Geometry: final body of the model. Coordinates: model frame, mm. Face numbers are marked on the shaded views. Round coordinates to 2 decimals unless told otherwise and drop trailing zeros. Write each loop counter-clockwise with the first axis right and the second up, starting at its lowest first coordinate (ties: lowest second). Pieces come first, ordered by that corner, then holes. Notation, with made-up numbers: (-33.5, 8.5) - (-9.5, 8.5) arc R17 cw to (-9.5, 28.5) - close; hole circle Ø9 at (15, -35.5). An arc over 180 degrees is marked (long way). Write each question's results on one line, items separated by ' | '.
from build123d import *

# Parameters (mm, degrees)
SKETCH_1_W          = 268
SKETCH_1_H          = 150
EXTRUDE_1_DEPTH     = 12
SKETCH_2_W          = 258
SKETCH_2_H          = 150
CUT_EXTRUDE_1_DEPTH = 2
CUT_EXTRUDE_2_DEPTH = 154.886321679
HOLE_WIZARD_M6_1_D  = 5
CHAMFER_1_SIZE      = 3


with BuildPart() as part:
    # 草图1 → 凸台-拉伸1 (new body)
    with BuildSketch(Plane.XY):
        Rectangle(SKETCH_1_W, SKETCH_1_H)
    extrude(amount=EXTRUDE_1_DEPTH)

    # 草图2 → 切除-拉伸1 (cut)
    with BuildSketch(Plane.XY.offset(12)):
        Rectangle(SKETCH_2_W, SKETCH_2_H)
    extrude(amount=-CUT_EXTRUDE_1_DEPTH, mode=Mode.SUBTRACT)

    # 草图3 → 切除-拉伸2 (cut, through all)
    with BuildSketch(Plane.XY.offset(10)):
        with BuildLine():
            Line((-80, 53.3), (-50, 53.3))
            ThreePointArc((-50, 53.3), (-46.7, 50), (-50, 46.7))
            Line((-50, 46.7), (-80, 46.7))
            ThreePointArc((-80, 46.7), (-83.3, 50), (-80, 53.3))
        make_face()
        with BuildLine():
            Line((50, 53.3), (80, 53.3))
            ThreePointArc((80, 53.3), (83.3, 50), (80, 46.7))
            Line((80, 46.7), (50, 46.7))
            ThreePointArc((50, 46.7), (46.7, 50), (50, 53.3))
        make_face()
        with BuildLine():
            Line((-80, -46.7), (-50, -46.7))
            ThreePointArc((-50, -46.7), (-46.7, -50), (-50, -53.3))
            Line((-50, -53.3), (-80, -53.3))
            ThreePointArc((-80, -53.3), (-83.3, -50), (-80, -46.7))
        make_face()
        with BuildLine():
            Line((50, -46.7), (80, -46.7))
            ThreePointArc((80, -46.7), (83.3, -50), (80, -53.3))
            Line((80, -53.3), (50, -53.3))
            ThreePointArc((50, -53.3), (46.7, -50), (50, -46.7))
        make_face()
    extrude(amount=-CUT_EXTRUDE_2_DEPTH, mode=Mode.SUBTRACT)

    # M6 螺纹孔1 (through all)
    with Locations(Plane.XY.offset(10)):
        with Locations((-119, 32.5), (-119, -32.5), (119, 32.5), (119, -32.5)):
            Hole(HOLE_WIZARD_M6_1_D / 2)

    # 倒角1
    chamfer_1_edges = [part.edges().sort_by_distance(p)[0] for p in [
        (134, -75, 6),
        (-134, -75, 6),
        (-134, 75, 6),
        (134, 75, 6),
    ]]
    chamfer(chamfer_1_edges, length=CHAMFER_1_SIZE)


solid = part.part
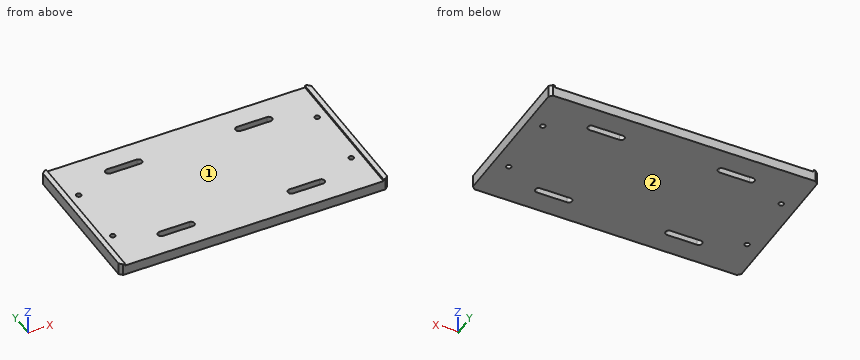
Q1. Pin query (flat end, axial travel): pin 1 (12 mm diameter, centred on x = 18.5, y = -22, fed in from +Z); pin 2 (4 mm diameter, centred on x = -119, y = -32.5, fed in from -Z). Return the tip coordinate at first contact, or that it passes through.
Answer block:
pin 1: z = 10 | pin 2: through
Q2. Section query B-B, the plane x = 119. Return loops of the section in (y, z).
Answer block:
outline: (-75, 0) - (-35, 0) - (-35, 10) - (-75, 10) - close; (-30, 0) - (30, 0) - (30, 10) - (-30, 10) - close; (35, 0) - (75, 0) - (75, 10) - (35, 10) - close
Q3. Ray query, line 1 along Y through (x, z) = (119, 4); line 2 along Y through (x, z) = (62, 5.75); line 3 along X through (y, z) = (-51.5, 8.5). Return the intervals inside material, ascending.
Answer block:
line 1: -75 to -35, -30 to 30, 35 to 75 | line 2: -75 to -53.3, -46.7 to 46.7, 53.3 to 75 | line 3: -134 to -82.94, -47.06 to 47.06, 82.94 to 134
Q4. Section query A-A, the plane y = -50. Return loops of the section in (x, z).
Answer block:
outline: (-134, 0) - (-83.3, 0) - (-83.3, 10) - (-129, 10) - (-129, 12) - (-134, 12) - close; (-46.7, 0) - (46.7, 0) - (46.7, 10) - (-46.7, 10) - close; (83.3, 0) - (134, 0) - (134, 12) - (129, 12) - (129, 10) - (83.3, 10) - close
Q5. Section query D-D, the plane y = 2. Return loops of the section in (x, z).
Answer block:
outline: (-134, 0) - (134, 0) - (134, 12) - (129, 12) - (129, 10) - (-129, 10) - (-129, 12) - (-134, 12) - close
Q6. Mould query, pull axis X, two halves, no side actions, for the marked faces 1 and 2. Classes: pulls with the +X half, pulls with the -X half, needs draft (parallel to the pull), parting line crosses it, or undercut.
Answer block:
face 1: undercut | face 2: needs draft
Q7. Section query C-C, the plane z = 2.5. Give the number of separate pieces and of enclosed holes in the cut face, plus the area to 3 significant figures.
Answer block:
separate pieces: 1 | enclosed holes: 8 | area: 39,200 mm2
